from build123d import *

# Parameters (mm, degrees)
SKETCH_1_W                = 26
SKETCH_1_H                = 12
EXTRUDE_1_DEPTH           = 5
HOLE_WIZARD_1_D           = 4.5
HOLE_WIZARD_1_CBORE_D     = 8
HOLE_WIZARD_1_CBORE_DEPTH = 4.6
HOLE_WIZARD_M6_1_D        = 5
CHAMFER_1_SIZE            = 0.5


with BuildPart() as part:
    # 草图1 → 凸台-拉伸1 (new, symmetric)
    with BuildSketch(Plane.XY):
        Rectangle(SKETCH_1_W, SKETCH_1_H)
    extrude(amount=EXTRUDE_1_DEPTH, both=True)

    # 打孔尺寸(%根据)内六角圆柱头螺钉的类型1 (through all)
    with Locations(Plane(origin=(0, 6, 0), x_dir=(1, 0, 0), z_dir=(0, 1, 0))):
        with Locations((-7.5, 0), (7.5, 0)):
            CounterBoreHole(HOLE_WIZARD_1_D / 2, HOLE_WIZARD_1_CBORE_D / 2, HOLE_WIZARD_1_CBORE_DEPTH)

    # M6 螺纹孔1 (through all)
    with Locations(Plane.XY.offset(5)):
        with Locations((0, 1)):
            Hole(HOLE_WIZARD_M6_1_D / 2)

    # 倒角1
    chamfer_1_edges = [part.edges().sort_by_distance(p)[0] for p in [
        (-13, 0, 5),
        (13, 0, 5),
        (-13, 0, -5),
        (13, 0, -5),
    ]]
    chamfer(chamfer_1_edges, length=CHAMFER_1_SIZE)


solid = part.part
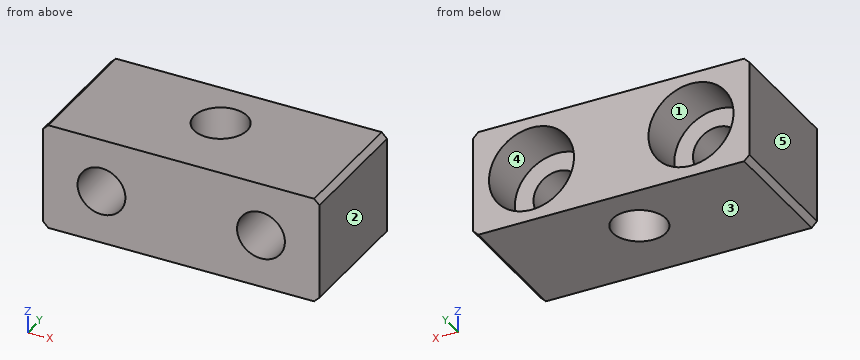
Verification items for the finished model (mm, model axes). Face numbers are marked on the shaded views. A direction names the side the tool comes from. Give positions to 0.01 mm unless a question says otherwise; leave off trailing zeros. Write each loop counter-clockwise with the first axis right and the second up, starting at its lowest first coordinate (ties: lowest second). Pieces come first, ordered by that corner, then holes. Notation, with made-up numbers: M 49,-4 L 80,-4 A13 ccw 80,0 Z; hole C -32.5,45.5 d3. An arc over 180 degrees is marked long. Write item = value, one per line.
(1) Go/stop test with flat-tipped pins: pin 1 Ø4 at (x, z) = (7.5, 0) entering from +Y; pin 2 Ø5 at (x, z) = (7.5, 0) entering from +Y. Record where each tip stops, or that it passes through.
Found:
pin_1 = through
pin_2 = 1.4
(2) Sectioned sample at D-D (y = 4.75). Record the cut outline in (x, z).
Found:
outline = M -13,-4.5 L -12.5,-5 L 12.5,-5 L 13,-4.5 L 13,4.5 L 12.5,5 L -12.5,5 L -13,4.5 Z; hole C -7.5,0 d8; hole C 7.5,0 d8
(3) Sectioned sample at A-A (z = 0). Record the cut outline in (x, y).
Found:
outline = M -13,-6 L -9.75,-6 L -9.75,1.4 L -11.5,1.4 L -11.5,6 L -13,6 Z; M -5.25,-6 L 5.25,-6 L 5.25,1.4 L 3.5,1.4 L 3.5,6 L -3.5,6 L -3.5,1.4 L -5.25,1.4 Z; M 9.75,-6 L 13,-6 L 13,6 L 11.5,6 L 11.5,1.4 L 9.75,1.4 Z; hole C 0,1 d5
(4) Material ranges on line 1 (Z direction, x = 7.5, y = 4.2); line 2 (Y direction, x = 0, z = 1.5); line 3 (X direction, y = -5, z = -0.25), recorded low to high.
Found:
line_1 = -5 to -4, 4 to 5
line_2 = -6 to -1.5, 3.5 to 6
line_3 = -13 to -9.74, -5.26 to 5.26, 9.74 to 13
(5) Draft check along X on the marked faces 3, 4 and 5. Enter one of: released by +X, released by -X, zero draft, split by the parting line, or undercut.
Found:
face_3 = zero draft
face_4 = undercut
face_5 = released by -X
(6) Sectioned sample at B-B (y = -1). Record the cut outline in (x, z).
Found:
outline = M -13,-4.5 L -12.5,-5 L -1.5,-5 L -1.5,5 L -12.5,5 L -13,4.5 Z; M 1.5,-5 L 12.5,-5 L 13,-4.5 L 13,4.5 L 12.5,5 L 1.5,5 Z; hole C -7.5,0 d4.5; hole C 7.5,0 d4.5
(7) Sectioned sample at C-C (x = 7.5). Record the cut outline in (y, z), then the cut area to 3 significant figures.
Found:
outline = M -6,-5 L 6,-5 L 6,-4 L 1.4,-4 L 1.4,-2.25 L -6,-2.25 Z; M -6,2.25 L 1.4,2.25 L 1.4,4 L 6,4 L 6,5 L -6,5 Z
area = 49.9 mm2
(8) Access from +Z, -Z, +X, -X, +Y, -Y to the whole of each face (thin tool, end or side, straight path). Record for the marked faces 1 and 2.
Found:
face_1 = +Y
face_2 = +Z, -Z, +X, +Y, -Y
